Here's how the part is built. I have some questions about the finished solid (model axes, mm). Coordinates: 2 decimals unless noted, no trailing zeros. Write each loop counter-clockwise with the first axis right and the second up, starting at its lowest first coordinate (ties: lowest second). Pieces come first, ordered by that corner, then holes.
Item 1: Please list where these lines run through material, in increasing order: line 1 (Y direction, x = 0, z = 2.5); line 2 (X direction, y = -3, z = 1.5); line 3 (X direction, y = 1.5, z = 2.75).
Item 2: I want a section at A-A (y = 0). Please give me the cut outline in (x, z).
Item 3: If we mould it in two halves opening along Y, with no side actions, what happens to faces 1 (the face through (-10, 0, 3)), 2 (the face through (73.695, -1.532, 3.042)), 3 (the face through (71, 5, 6))? For each: pulls with the +Y half, pulls with the -Y half, needs draft (parallel to the pull), parting line crosses it, or undercut.
Item 4: I want a section at B-B (z = 2.55). Please give me the cut outline in (x, y), and give its area (3 significant figures).
Item 5: I'm going to push flat-ended pins straight in: P1, Ø2, axis at y = 3.5, z = 5, coming from the -X side; P2, Ø5, axis at x = 70, y = 0, coming from the +Z side; P3, Ø1.5, axis at y = 3, z = 1, coming from the +X side. Where does each tip first touch, or does it pass through?
from build123d import *

# Parameters (mm, degrees)
BOSS_EXTRUDE1_DEPTH = 6
SKETCH2_R           = 4
CUT_EXTRUDE1_DEPTH  = 95
SKETCH3_R           = 4
CUT_EXTRUDE2_DEPTH  = 10


with BuildPart() as part:
    # Sketch1 → Boss-Extrude1 (new body)
    with BuildSketch(Plane.XY):
        with BuildLine():
            Line((0, 10), (140, 10))
            ThreePointArc((140, 10), (150, 0), (140, -10))
            Line((140, -10), (0, -10))
            ThreePointArc((0, -10), (-10, 0), (0, 10))
        make_face()
    extrude(amount=BOSS_EXTRUDE1_DEPTH)

    # Sketch2 → Cut-Extrude1 (cut)
    with BuildSketch(Plane.XY.offset(6)):
        Circle(SKETCH2_R)
        with Locations((140, 0)):
            Circle(SKETCH2_R)
    extrude(amount=-CUT_EXTRUDE1_DEPTH, mode=Mode.SUBTRACT)

    # Sketch3 → Cut-Extrude2 (cut)
    with BuildSketch(Plane.XY.offset(6)):
        with Locations((70, 0)):
            Circle(SKETCH3_R)
    extrude(amount=-CUT_EXTRUDE2_DEPTH, mode=Mode.SUBTRACT)


solid = part.part
Answer:
1. line 1: y = -10 to -4, 4 to 10
1. line 2: x = -9.54 to -2.65, 2.65 to 67.35, 72.65 to 137.35, 142.65 to 149.54
1. line 3: x = -9.89 to -3.71, 3.71 to 66.29, 73.71 to 136.29, 143.71 to 149.89
2. outline: (-10, 0) - (-4, 0) - (-4, 6) - (-10, 6) - close; (4, 0) - (66, 0) - (66, 6) - (4, 6) - close; (74, 0) - (136, 0) - (136, 6) - (74, 6) - close; (144, 0) - (150, 0) - (150, 6) - (144, 6) - close
3. face 1: parting line crosses it
3. face 2: undercut
3. face 3: needs draft
4. outline: (0, -10) - (140, -10) arc R10 ccw to (140, 10) - (0, 10) arc R10 ccw to start; hole circle Ø8 at (0, 0); hole circle Ø8 at (70, 0); hole circle Ø8 at (140, 0)
4. area: 2,960 mm2
5. P1: stops at x = -9.68
5. P2: passes through
5. P3: stops at x = 149.74
